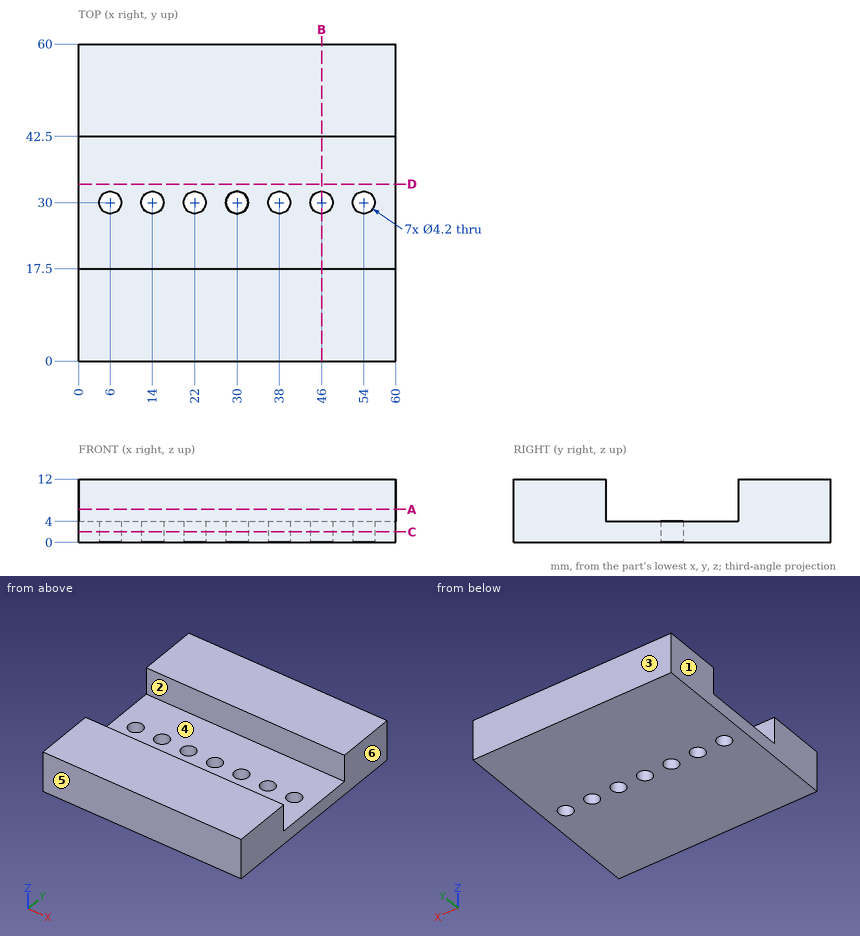
Print and shaded views of the part. All mm, measured from the part's lowest x, y and z. A direction names the side the tool comes from. Coordinates: 2 decimals unless noted, no trailing zeros. Loops run counter-clockwise (first coordinate to the right, second up) from the corner with the lowest first, then second, coordinate; pieces in that order, holes last. Notation, with made-up numbers: (44.5, 22.25) -> (50.5, 22.25) arc R12 cw to (50.5, 40.25) -> close; hole circle Ø3 at (-9, 0). An arc over 180 degrees is marked (long way). Use a Markdown table: item, result. Add a question column.
Item 1: Flat gauge pins, fed straight in: P1, Ø7.5, axis at x = 19.5, y = 25.5, coming from the +Z side; P2, Ø6, axis at x = 38, y = 41, coming from the +Z side. Where does each tip first touch, or does it go through?
Item 2: Band-saw the part on B-B on x = 46. Write the cut outline in (y, z).
Item 3: Pull direction Y, two halves, no side cores. Call the marked faces 3, 4, 5 and 6: +Y half, -Y half, draft (parallel to the pull), parting line (faces both ways), or undercut.
Item 4: Band-saw the part on D-D on y = 33.5. Write the cut outline in (x, z).
Item 5: Band-saw the part on A-A on z = 6.25. Write the cut outline in (x, y).
Item 6: Which spindle directions (+Z, -Z, +X, -X, +Y, -Y) get a long thin tool onto all of the face, cutting with end or side? Do the marked faces 1 and 2. Say none if no direction does.
Item 7: Probe probe 1 along Y at (x, z) = (24, 4.25); probe 2 along Y at (x, z) = (22, 1.75); probe 3 along Z at (x, y) = (7, 35.5). List the from-to ranges inside material, lowest first.
Item 8: Band-saw the part on C-C on z = 2. Write the cut outline in (x, y).
Geometry says:
| question | item | result |
|---|---|---|
| 1 | P1 | z = 4 |
| 1 | P2 | z = 12 |
| 2 | outline | (0, 0) -> (27.9, 0) -> (27.9, 4) -> (17.5, 4) -> (17.5, 12) -> (0, 12) -> close; (32.1, 0) -> (60, 0) -> (60, 12) -> (42.5, 12) -> (42.5, 4) -> (32.1, 4) -> close |
| 3 | face 3 | +Y half |
| 3 | face 4 | undercut |
| 3 | face 5 | -Y half |
| 3 | face 6 | draft |
| 4 | outline | (0, 0) -> (60, 0) -> (60, 4) -> (0, 4) -> close |
| 5 | outline | (0, 0) -> (60, 0) -> (60, 17.5) -> (0, 17.5) -> close; (0, 42.5) -> (60, 42.5) -> (60, 60) -> (0, 60) -> close |
| 6 | face 1 | +Z, -Z, -X, +Y, -Y |
| 6 | face 2 | +Z, +X, -X |
| 7 | probe 1 | 0 to 17.5, 42.5 to 60 |
| 7 | probe 2 | 0 to 27.9, 32.1 to 60 |
| 7 | probe 3 | 0 to 4 |
| 8 | outline | (0, 0) -> (60, 0) -> (60, 60) -> (0, 60) -> close; hole circle Ø4.2 at (6, 30); hole circle Ø4.2 at (14, 30); hole circle Ø4.2 at (22, 30); hole circle Ø4.2 at (30, 30); hole circle Ø4.2 at (38, 30); hole circle Ø4.2 at (46, 30); hole circle Ø4.2 at (54, 30) |
